```python
from build123d import *


with BuildPart() as part:
    # Sketch2 → Revolve1 (revolve)
    with BuildSketch(Plane(origin=(0, 0, 0), x_dir=(0, 0, -1), z_dir=(1, 0, 0)), mode=Mode.PRIVATE) as revolve1_sk:
        Polygon((0, 17.5), (0, 12), (1.25, 12), (3.000518846, 9.5), (23, 9.5), (38, 14), (38, 22), (20, 22), (20, 26), (15, 26), (15, 14.5), (12.5, 14.5), (12.5, 17.5), align=None)
    revolve(revolve1_sk.sketch.rotate(Axis((0, 0, 28.492460363), (0, 0, -1)), 90), axis=Axis((0, 0, 28.492460363), (0, 0, -1)))


solid = part.part
```
Here's how the part is built. I have some questions about the finished solid (model axes, mm). A direction names the side the tool comes from. Coordinates: 2 decimals unless noted, no trailing zeros. Write each loop counter-clockwise with the first axis right and the second up, starting at its lowest first coordinate (ties: lowest second). Pieces come first, ordered by that corner, then holes. Notation, with made-up numbers: (37.5, -27.5) -> (71.5, -27.5) arc R21 cw to (71.5, -11.5) -> close; hole circle Ø5 at (72.25, 76). An arc over 180 degrees is marked (long way). Use a Markdown table: item, result. Add a question column.
(1) For faces 4 (the cylindrical face through (6.691, 12.864, -13.732)), 5 (the flat face through (-12, 4, 0)), 6 (the cylindrical face through (11.446, -3.604, -0.634)), 7 (the flat face through (19, -12, -20)), which set-ups out of +Z, -Z, +X, -X, +Y, -Y let a thin tool reach every point of the face, with its end or its side?
(2) Please list where these lines run through material, in increasing order: line 1 (Z direction, x = -8, y = -13); line 2 (Z direction, x = 19, y = 7.5); line 3 (Y direction, x = 0, z = -9.25).
(3) If we section it at C-C, the plane y = 20: Write out the boundary of the cut face in (x, z), and give its area (3 significant figures).
(4) If we section it at A-A, the plane x = 0: Write out the boundary of the cut face in (y, z).
(5) If we section it at D-D, the plane z = -32: Write out the boundary of the cut face in (x, y).
(6) I'm going to push flat-ended pins straight in: P1, Ø5, axis at y = -2, z = -10.5, coming from the +X side; P2, Ø10, axis at y = 4.5, z = -29.5, coming from the -X side; P3, Ø1.5, axis at y = 0.5, z = -24, coming from the +X side. Where does each tip first touch, or does it pass through?
(7) We'd pull the mould along Y, two halves only. Please class faces 1 (the cylindrical face through (-4.769, 21.477, -28.874)), 2 (the conical face through (-2.337, 10.525, -27.272)), 3 (the flat face through (7, -13, -12.5)): +Y half, -Y half, draft (parallel to the pull), parting line (faces both ways), or undercut.
Outcome:
| question | item | result |
|---|---|---|
| 1 | face 4 | none |
| 1 | face 5 | +Z, +X, -X, +Y, -Y |
| 1 | face 6 | +Z |
| 1 | face 7 | -Z |
| 2 | line 1 | z = -38 to -15, -12.5 to 0 |
| 2 | line 2 | z = -38 to -15 |
| 2 | line 3 | y = -17.5 to -9.5, 9.5 to 17.5 |
| 3 | outline | (-16.61, -20) -> (-9.17, -20) -> (-9.17, -38) -> (9.17, -38) -> (9.17, -20) -> (16.61, -20) -> (16.61, -15) -> (-16.61, -15) -> close |
| 3 | area | 496 mm^2 |
| 4 | outline | (-26, -20) -> (-22, -20) -> (-22, -38) -> (-14, -38) -> (-9.5, -23) -> (-9.5, -3) -> (-12, -1.25) -> (-12, 0) -> (-17.5, 0) -> (-17.5, -12.5) -> (-14.5, -12.5) -> (-14.5, -15) -> (-26, -15) -> close; (9.5, -23) -> (14, -38) -> (22, -38) -> (22, -20) -> (26, -20) -> (26, -15) -> (14.5, -15) -> (14.5, -12.5) -> (17.5, -12.5) -> (17.5, 0) -> (12, 0) -> (12, -1.25) -> (9.5, -3) -> close |
| 5 | outline | circle Ø44 at (0, 0); hole circle Ø24.4 at (0, 0) |
| 6 | P1 | stops at x = 17.5 |
| 6 | P2 | stops at x = -22 |
| 6 | P3 | stops at x = 22 |
| 7 | face 1 | parting line |
| 7 | face 2 | undercut |
| 7 | face 3 | draft |
